```python
from build123d import *

# Parameters (mm, degrees)
SKETCH1_R           = 95
BOSS_EXTRUDE1_DEPTH = 600
SKETCH2_R           = 50
BOSS_EXTRUDE2_DEPTH = 10
BOSS_EXTRUDE3_START = 10
SKETCH3_R           = 50
BOSS_EXTRUDE3_DEPTH = 10
SKETCH4_R           = 27.5
BOSS_EXTRUDE4_DEPTH = 20
BOSS_EXTRUDE5_START = 20
SKETCH5_R           = 27.5
BOSS_EXTRUDE5_DEPTH = 20


with BuildPart() as part:
    # Sketch1 → Boss-Extrude1 (new body)
    with BuildSketch(Plane.XY):
        Circle(SKETCH1_R)
    extrude(amount=BOSS_EXTRUDE1_DEPTH)

    # Sketch2 → Boss-Extrude2 (add)
    with BuildSketch(Plane.XY.offset(600)):
        Circle(SKETCH2_R)
    extrude(amount=BOSS_EXTRUDE2_DEPTH)

    # Sketch3 → Boss-Extrude3 (add)
    with BuildSketch(Plane(origin=(0, 0, 0), x_dir=(-1, 0, 0), z_dir=(0, 0, -1)).offset(BOSS_EXTRUDE3_START)):
        with Locations(Location((0, 0, 0), (0, 0, 180))):
            Circle(SKETCH3_R)
    extrude(amount=-BOSS_EXTRUDE3_DEPTH)

    # Sketch4 → Boss-Extrude4 (add)
    with BuildSketch(Plane(origin=(0, 0, -10), x_dir=(-1, 0, 0), z_dir=(0, 0, -1))):
        Circle(SKETCH4_R)
    extrude(amount=BOSS_EXTRUDE4_DEPTH)

    # Sketch5 → Boss-Extrude5 (add)
    with BuildSketch(Plane.XY.offset(610).offset(BOSS_EXTRUDE5_START)):
        with Locations(Location((0, 0, 0), (0, 0, 180))):
            Circle(SKETCH5_R)
    extrude(amount=-BOSS_EXTRUDE5_DEPTH)


solid = part.part
```
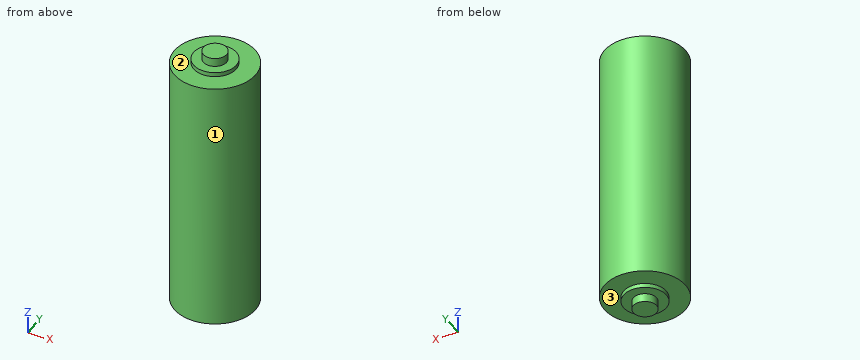
Geometry check sheet. Reference: the model listing, model coordinates, mm. Face numbers are marked on the shaded views. A direction names the side the tool comes from. Coordinates: 2 decimals unless noted, no trailing zeros. Write each loop counter-clockwise with the first axis right and the second up, starting at its lowest first coordinate (ties: lowest second). Pieces come first, ordered by that corner, then holes. Notation, with made-up numbers: M 30.25,-2 L 66.25,-2 A12 cw 66.25,7 Z; hole C 43,39.25 d11. An arc over 180 degrees is marked long. One line per item, written item: value. Start each with the question number.
(1) Depth check by flat-ended pin: pin 1 (1.5 mm diameter, centred on y = 32, z = 163, fed in from +X); pin 2 (12 mm diameter, centred on x = -46, y = 21.5, fed in from -Z); pin 3 (3 mm diameter, centred on y = 25, z = 106.5, fed in from -X); pin 4 (12 mm diameter, centred on x = -27, y = -16, fed in from +Z). Enter the tip coordinate at first touch or a pass-through.
(2) Scan lines: line 1 along Z through (x, y) = (50.5, 41.5); line 2 along Y through (x, z) = (-2.5, 323); line 3 along Z through (x, y) = (41, 13). Record each from-to range of solid material in increasing order. Write a range as [from, to].
(3) Sectioned sample at D-D, the plane x = 36.5. Enter the section's corners in (y, z), and give its area (3 significant figures).
(4) Tool access check on the marked faces 1, 2 and 3. Record the directions out of +Z, -Z, +X, -X, +Y, -Y that give a thin tool (end or side, any length) a straight path to the whole face; none if there is none.
(5) Sectioned sample at A-A, the plane y = 0. Enter the section's corners in (x, z).
(6) Sectioned sample at C-C, the plane z = 499.5. Enter the section's corners in (x, y), and give its area (3 significant figures).
Filled sheet:
1. pin 1: x = 89.71
1. pin 2: z = -10
1. pin 3: x = -92.05
1. pin 4: z = 630
2. line 1: [0, 600]
2. line 2: [-94.97, 94.97]
2. line 3: [-10, 610]
3. outline: M -87.71,0 L -34.17,0 L -34.17,-10 L 34.17,-10 L 34.17,0 L 87.71,0 L 87.71,600 L 34.17,600 L 34.17,610 L -34.17,610 L -34.17,600 L -87.71,600 Z
3. area: 107,000 mm²
4. face 1: +Z, -Z
4. face 2: +Z
4. face 3: -Z
5. outline: M -95,0 L -50,0 L -50,-10 L -27.5,-10 L -27.5,-30 L 27.5,-30 L 27.5,-10 L 50,-10 L 50,0 L 95,0 L 95,600 L 50,600 L 50,610 L 27.5,610 L 27.5,630 L -27.5,630 L -27.5,610 L -50,610 L -50,600 L -95,600 Z
6. outline: C 0,0 d190
6. area: 28,400 mm²
